Build history of the part. All positions in model axes, mm. A direction names the side the tool comes from. Round coordinates to 2 decimals unless told otherwise and drop trailing zeros. Write each loop counter-clockwise with the first axis right and the second up, starting at its lowest first coordinate (ties: lowest second). Pieces come first, ordered by that corner, then holes. Notation, with made-up numbers: (-24.75, 18.25) -> (-14.75, 18.25) arc R30 ccw to (-14.75, 40.25) -> close; hole circle Ø7 at (-1.5, -20.5). An arc over 180 degrees is marked (long way). Answer as CSV lines item,"result".
from build123d import *

# Parameters (mm, degrees)
SKETCH2_W           = 6
SKETCH2_H           = 6
BOSS_EXTRUDE1_DEPTH = 2
BOSS_EXTRUDE2_START = 32
SKETCH3_R           = 3
BOSS_EXTRUDE2_DEPTH = 32
CUT_EXTRUDE2_START  = 3
CUT_EXTRUDE2_DEPTH  = 1.6
CUT_EXTRUDE3_START  = -1.4
CUT_EXTRUDE3_DEPTH  = 1.6


with BuildPart() as part:
    # Sketch1 → Revolve1 (revolve)
    with BuildSketch(Plane.XY, mode=Mode.PRIVATE) as revolve1_sk:
        Polygon((0, 0), (3, 0), (3, 4.95), (6, 4.95), (6, 5.95), (0, 5.95), align=None)
    revolve(revolve1_sk.sketch.rotate(Axis((0, -2.859551482, 0), (0, 1, 0)), 90), axis=Axis((0, -2.859551482, 0), (0, 1, 0)))

    # Sketch2 → Boss-Extrude1 (add)
    with BuildSketch(Plane(origin=(0, 5.95, 0), x_dir=(1, 0, 0), z_dir=(0, 1, 0))):
        Rectangle(SKETCH2_W, SKETCH2_H)
    extrude(amount=BOSS_EXTRUDE1_DEPTH)

    # Sketch3 → Boss-Extrude2 (add)
    with BuildSketch(Plane(origin=(0, 7.95, 0), x_dir=(1, 0, 0), z_dir=(0, 1, 0)).offset(BOSS_EXTRUDE2_START)):
        with Locations(Location((0, 0, 0), (0, 0, 90))):
            Circle(SKETCH3_R)
    extrude(amount=-BOSS_EXTRUDE2_DEPTH)

    # Sketch 4_2 → Cut-Extrude2 (cut)
    with BuildSketch(Plane.XY.offset(CUT_EXTRUDE2_START)):
        with BuildLine():
            Line((-2, 32.95), (-2, 34.95))
            ThreePointArc((-2, 34.95), (0, 36.95), (2, 34.95))
            Line((2, 34.95), (2, 32.95))
            ThreePointArc((2, 32.95), (0, 30.95), (-2, 32.95))
        make_face()
    extrude(amount=-CUT_EXTRUDE2_DEPTH, mode=Mode.SUBTRACT)

    # Sketch 4_2 2 → Cut-Extrude3 (cut)
    with BuildSketch(Plane.XY.offset(CUT_EXTRUDE3_START)):
        with BuildLine():
            Line((-2, 32.95), (-2, 34.95))
            ThreePointArc((-2, 34.95), (0, 36.95), (2, 34.95))
            Line((2, 34.95), (2, 32.95))
            ThreePointArc((2, 32.95), (0, 30.95), (-2, 32.95))
        make_face()
    extrude(amount=-CUT_EXTRUDE3_DEPTH, mode=Mode.SUBTRACT)


solid = part.part
1. Drop flat-ended pins along their axis: pin 1 Ø2 at (x, z) = (-4, -1) entering from -Y; pin 2 Ø1.2 at (x, y) = (-1, 35) entering from -Z; pin 3 Ø5 at (y, z) = (27.5, 3) entering from -X. Give the stop position or say it passes through.
Results found:
pin 1,"stops at y = 4.95"
pin 2,"stops at z = -1.4"
pin 3,"stops at x = -2.96"
2. Cut at A-A, the plane y = 34. Write the cut outline in (x, z), then the cut area to 3 significant figures.
Results found:
outline,"(-2, -2.24) -> (-2, -1.4) -> (2, -1.4) -> (2, -2.24) arc R3 ccw to (2, 2.24) -> (2, 1.4) -> (-2, 1.4) -> (-2, 2.24) arc R3 ccw to start"
area,"17.4 mm2"
3. Which spindle directions (+Z, -Z, +X, -X, +Y, -Y) get a long thin tool onto all of the face, cutting with end or side? Do faces 1 (the flat face through (0, 34, 1.4)), 2 (the flat face through (-3, 4.95, 1)), 3 (the cylindrical face through (-3, 24, 0)). Say none if no direction does.
Results found:
face 1,"+Z"
face 2,"-Y"
face 3,"+Y"
4. Cut at D-D, the plane y = 4. Write the cut outline in (x, z).
Results found:
outline,"circle Ø6 at (0, 0)"
5. Mould opens along Y. For faces 4 (the cylindrical face through (0.04, 30.95, 2.03)), 5 (the cylindrical face through (-1.802, 5.457, -5.723)), 6 (the flat face through (-2.4, 7.95, -2.3)), 7 (the cylindrical face through (-0.04, 36.95, -2.01)) say: +Y half, -Y half, draft (parallel to the pull), parting line (faces both ways), or undercut.
Results found:
face 4,"undercut"
face 5,"draft"
face 6,"+Y half"
face 7,"undercut"
6. Cut at C-C, the plane z = -3.5. Write the cut outline in (x, y).
Results found:
outline,"(-4.87, 4.95) -> (4.87, 4.95) -> (4.87, 5.95) -> (-4.87, 5.95) -> close"
7. Cut at B-B, the plane x = 1.5. Write the cut outline in (y, z), then the cut area to 3 significant figures.
Results found:
outline,"(0, -2.6) -> (4.95, -2.6) -> (4.95, -5.81) -> (5.95, -5.81) -> (5.95, -3) -> (7.95, -3) -> (7.95, -2.6) -> (31.63, -2.6) -> (31.63, -1.4) -> (36.27, -1.4) -> (36.27, -2.6) -> (39.95, -2.6) -> (39.95, 2.6) -> (36.27, 2.6) -> (36.27, 1.4) -> (31.63, 1.4) -> (31.63, 2.6) -> (7.95, 2.6) -> (7.95, 3) -> (5.95, 3) -> (5.95, 5.81) -> (4.95, 5.81) -> (4.95, 2.6) -> (0, 2.6) -> close"
area,"204 mm2"
8. Probe line 1 along Y through (x, z) = (4.75, 0.5); line 2 along X through (y, z) = (6, 1); line 3 along X through (y, z) = (21, 1.75). List the from-to ranges inside material, lowest first.
Results found:
line 1,"y = 4.95 to 5.95"
line 2,"x = -3 to 3"
line 3,"x = -2.44 to 2.44"
